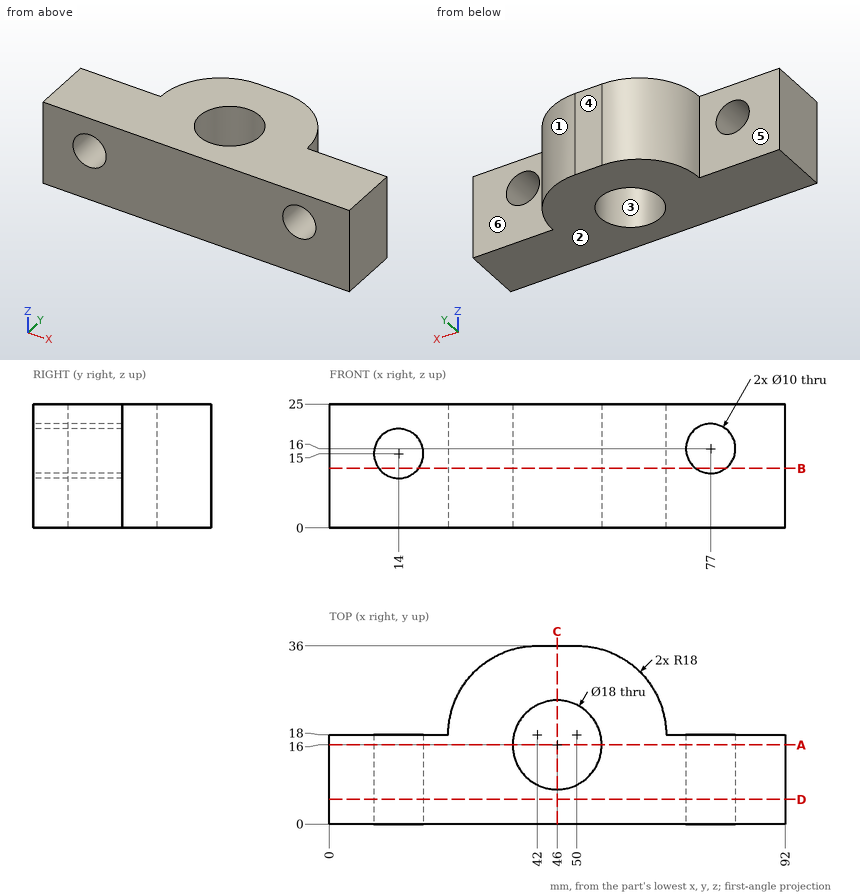
Study the drawing (mm; zero at the part's minimum x, y, z) and answer. A direction names the side the tool comes from. Round coordinates to 2 decimals unless told otherwise and drop trailing zeros. Order: outer loops, then holes, each group sorted by start corner. A loop starts at its lowest first (then second) coordinate and runs counter-clockwise, first axis right, second up. Notation, with made-up numbers: M 55.25,54.5 L 99.25,54.5 A17 cw 99.25,71.5 Z; hole C -17,68.25 d8. An arc over 180 degrees is marked long. One line per item, written item: value.
Q1. Straight lines are drawn through the part: line 1 (Z direction, x = 77, y = 11.25); line 2 (X direction, y = 13.5, z = 16); line 3 (Z direction, x = 14, y = 6.25). For each, find the intervals that lie inside material, in ascending order.
Derived:
line 1: 0 to 11, 21 to 25
line 2: 0 to 9.1, 18.9 to 37.35, 54.65 to 72, 82 to 92
line 3: 0 to 10, 20 to 25
Q2. For the marked faces 4, 5 and 6, determine the directions among +Z, -Z, +X, -X, +Y, -Y from which every point of the face is accessible in a straight line to the end or side of a thin tool.
Derived:
face 4: +Z, -Z, +X, -X, +Y
face 5: +Z, -Z, -X, +Y
face 6: +Z, -Z, +X, +Y
Q3. Find section C-C on x = 46. Write down the section's boundary in (y, z).
Derived:
outline: M 0,0 L 7,0 L 7,25 L 0,25 Z; M 25,0 L 36,0 L 36,25 L 25,25 Z
Q4. Find section D-D on y = 5. Write down the section's boundary in (x, z), then the cut area to 3 significant figures.
Derived:
outline: M 0,0 L 92,0 L 92,25 L 0,25 Z; hole C 14,15 d10; hole C 77,16 d10
area: 2,140 mm²
Q5. Flat-ended cylindrical pins translate along their axes: pin 1 (7 mm diameter, centred on x = 80.5, z = 15.5, fed in from +Y); pin 2 (4 mm diameter, centred on x = 31, z = 15, fed in from +Y); pin 3 (1 mm diameter, centred on x = 41.5, y = 23, fed in from +Z); pin 4 (6 mm diameter, centred on y = 26.5, z = 19, fed in from -X). Find the tip coordinate at first contact, or state that the pin passes through.
Derived:
pin 1: y = 18
pin 2: y = 33.59
pin 3: through
pin 4: x = 24.86
Q6. Find section B-B on z = 12. Write down the section's boundary in (x, y).
Derived:
outline: M 0,0 L 10,0 L 10,18 L 0,18 Z; M 18,0 L 74,0 L 74,18 L 68,18 A18 ccw 50,36 L 42,36 A18 ccw 24,18 L 18,18 Z; M 80,0 L 92,0 L 92,18 L 80,18 Z; hole C 46,16 d18
Q7. Determine the mould class of the marked faces 1, 2 and 3 for opening direction X: released by +X, released by -X, zero draft, split by the parting line, or undercut.
Derived:
face 1: released by +X
face 2: zero draft
face 3: undercut
Q8. Find section A-A on y = 16. Write down the section's boundary in (x, z).
Derived:
outline: M 0,0 L 37,0 L 37,25 L 0,25 Z; M 55,0 L 92,0 L 92,25 L 55,25 Z; hole C 14,15 d10; hole C 77,16 d10
